Study the drawing (mm; zero at the part's minimum x, y, z) and answer. A direction names the side the tool comes from. Coordinates: 2 decimals unless noted, no trailing zeros. Loops run counter-clockwise (first coordinate to the right, second up) from the corner with the lowest first, then second, coordinate; pieces in that order, holes last. Notation, with made-up numbers: (-37, 22.25) - (-19, 22.25) arc R27 ccw to (-19, 52.25) - close; hole circle Ø1 at (26.5, 34). An arc over 180 degrees is marked (long way). Use CSV: the item, a comma, the result in double quotes.
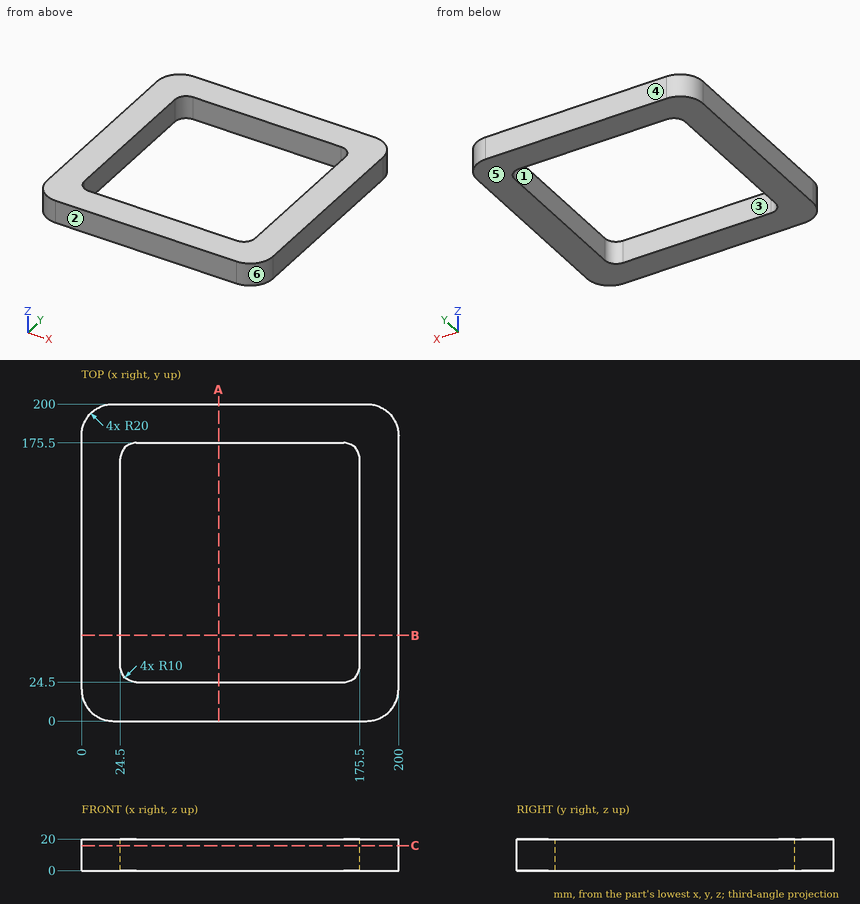
Q1. Given P1, Ø5, axis at x = 160.5, y = 172, coming from the +Z side, flat-ended and moving along its own axis, determine where the tip first touches the part or whether it passes through.
Reported:
P1,"passes through"
Q2. The part is cut by section A-A on x = 86.5. Determine the outline of the cut face in (y, z), and give its area (3 significant figures).
Reported:
outline,"(0, 0) - (24.5, 0) - (24.5, 20) - (0, 20) - close; (175.5, 0) - (200, 0) - (200, 20) - (175.5, 20) - close"
area,"980 mm²"
Q3. A tool of negligible diameter and unlimited length cuts with its end or side. For the marked faces 1 and 2, from which of +Z, -Z, +X, -X, +Y, -Y can it reach the whole face along a straight path? Write none if from no direction.
Reported:
face 1,"+Z, -Z"
face 2,"+Z, -Z, +X, -X, -Y"
Q4. Find the intervals of material crossed by probe 1 along X at (y, z) = (124, 11.25); probe 2 along X at (y, z) = (32, 5), in increasing order. Write a range as [from, to].
Reported:
probe 1,"x = [0, 24.5], [175.5, 200]"
probe 2,"x = [0, 24.82], [175.18, 200]"
Q5. For a pull along Y with two mould halves and no side action, classify the marked faces 3, 4, 5 and 6 as +Y half, -Y half, draft (parallel to the pull), parting line (faces both ways), or undercut.
Reported:
face 3,"undercut"
face 4,"+Y half"
face 5,"draft"
face 6,"-Y half"
Q6. The part is cut by section C-C on z = 15.75. Determine the outline of the cut face in (x, y), and give its area (3 significant figures).
Reported:
outline,"(0, 20) arc R20 ccw to (20, 0) - (180, 0) arc R20 ccw to (200, 20) - (200, 180) arc R20 ccw to (180, 200) - (20, 200) arc R20 ccw to (0, 180) - close; hole (24.5, 34.5) arc R10 ccw to (34.5, 24.5) - (165.5, 24.5) arc R10 ccw to (175.5, 34.5) - (175.5, 165.5) arc R10 ccw to (165.5, 175.5) - (34.5, 175.5) arc R10 ccw to (24.5, 165.5) - close"
area,"16,900 mm²"
